The model under review builds one solid part; all positions refer to its coordinate system, in mm. A direction names the side the tool comes from. Round coordinates to 2 decimals unless told otherwise and drop trailing zeros. Write each loop counter-clockwise with the first axis right and the second up, starting at its lowest first coordinate (ties: lowest second). Pieces come first, ordered by that corner, then holes. Notation, with made-up numbers: (-6, 63.25) -> (6, 63.25) arc R28 cw to (6, 99.25) -> close; hole circle Ø7 at (80.25, 84). An arc over 180 degrees is marked (long way). Answer as a JSON object with one key per item and string values. Group by question number.
1) Machinability: for faces 5 (the cylindrical face through (68.476, -39.816, 4.336)), 6 (the cylindrical face through (55.99, -52.58, 16.85)), 7 (the cylindrical face through (4.056, 38.668, 5.077)), which of the approach directions +Z, -Z, +X, -X, +Y, -Y give a long, thin tool a straight path to every point of the face, cutting with its end or side? Answer none if there is none.
2) We need section C-C, the plane z = -29.5. Write out the cut boundary in (x, y).
3) Mouldability with a two-part tool opening along X and no side actions: class faces 1 (the cylindrical face through (55.844, -52.577, -16.716)), 2 (the cylindrical face through (75.31, -46.66, 2.82)), 3 (the cylindrical face through (132, -53, 0)), 4 (the flat face through (87, -47, 24)) as pulls with the +X half, pulls with the -X half, needs draft (parallel to the pull), parting line crosses it, or undercut.
4) We need section B-B, the plane x = 117. Write out the cut boundary in (y, z).
5) Insertion check: pin 1 Ø6 at (y, z) = (-30, 0) entering from -X; pin 2 Ø2 at (y, z) = (-43, -15) entering from +X; pin 3 Ø1.5 at (x, y) = (31, 12) entering from -Z. Each pin has a flat end and moves straight along its axis. Give the tip position at first contact, or say it passes through.
6) We need section D-D, the plane z = 0. Count the separate pieces of the cut face and the enclosed holes in it, then the cut area to 3 significant figures.
7) We need section A-A, the plane y = 30. Write out the cut boundary in (x, z).
8) To check wall thickness, follow probe 1 along Z at (x, y) = (88, -42.5); probe 2 along Y at (x, z) = (102, -19); probe 3 along Z at (x, y) = (94.5, -13). State the ranges of each line that lie inside material, in increasing order. Write a range as [from, to].
from build123d import *

# Parameters (mm, degrees)
PIPE_SECTION_SKETCH_40X_26_R        = 20
PIPE_SECTION_SKETCH_40X_26_R_2      = 13
ROUND_START                         = 8
ROUND_FLANGE_SKETCH_78_R            = 39
ROUND_FLANGE_SKETCH_78_R_2          = 13
ROUND_FLANGE_78_DEPTH               = 8
ROUND_FLANGE_BOLT_HOLES_4X_10_REACH = 130.643
ROUND_FLANGE_BOLT_HOLES_SKETCH_R    = 5
OVAL_FLANGE_SKETCH_R                = 6
OVAL_FLANGE_SKETCH_R_2              = 13
OVAL_FLANGE_DEPTH                   = 11
FLANGE_ROOT_FILLETS_R2_5_R          = 2.5


with BuildPart() as part:
    # Elbow Pipe Body: sweep along a path in Elbow Path Sketch
    with BuildLine(Plane.XY) as elbow_pipe_body_path:
        Line((0, 0), (53, 0))
        ThreePointArc((53, 0), (77.748737342, -10.251262658), (88, -35))
        Line((88, -35), (88, -58))
    # Pipe Section Sketch Ø40xØ26 → Elbow Pipe Body (sweep)
    with BuildSketch(Plane(origin=(0, 0, 0), x_dir=(0, 0, -1), z_dir=(1, 0, 0))):
        Circle(PIPE_SECTION_SKETCH_40X_26_R)
        Circle(PIPE_SECTION_SKETCH_40X_26_R_2, mode=Mode.SUBTRACT)
    sweep(path=elbow_pipe_body_path.line)

    # Round Flange Sketch Ø78 → Round Flange Ø78 (add)
    with BuildSketch(Plane(origin=(0, 0, 0), x_dir=(0, 0, -1), z_dir=(1, 0, 0)).offset(ROUND_START)):
        Circle(ROUND_FLANGE_SKETCH_78_R)
        with Locations(Location((0, 0, 0), (0, 0, 90))):
            Circle(ROUND_FLANGE_SKETCH_78_R_2, mode=Mode.SUBTRACT)
    extrude(amount=-ROUND_FLANGE_78_DEPTH)

    # Round Flange Bolt Holes Sketch → Round Flange Bolt Holes 4xØ10 (cut, up to next)
    with BuildSketch(Plane.ZY, mode=Mode.PRIVATE) as round_flange_bolt_holes_4x_10_sk1:
        with Locations((0, 30)):
            Circle(ROUND_FLANGE_BOLT_HOLES_SKETCH_R)
    round_flange_bolt_holes_4x_10_tool1 = extrude(round_flange_bolt_holes_4x_10_sk1.sketch, amount=-ROUND_FLANGE_BOLT_HOLES_4X_10_REACH, mode=Mode.PRIVATE) & part.part
    # Round Flange Bolt Holes Sketch → Round Flange Bolt Holes 4xØ10 (cut, up to next)
    with BuildSketch(Plane.ZY, mode=Mode.PRIVATE) as round_flange_bolt_holes_4x_10_sk2:
        with Locations((30, 0)):
            Circle(ROUND_FLANGE_BOLT_HOLES_SKETCH_R)
    round_flange_bolt_holes_4x_10_tool2 = extrude(round_flange_bolt_holes_4x_10_sk2.sketch, amount=-ROUND_FLANGE_BOLT_HOLES_4X_10_REACH, mode=Mode.PRIVATE) & part.part
    # Round Flange Bolt Holes Sketch → Round Flange Bolt Holes 4xØ10 (cut, up to next)
    with BuildSketch(Plane.ZY, mode=Mode.PRIVATE) as round_flange_bolt_holes_4x_10_sk3:
        with Locations((0, -30)):
            Circle(ROUND_FLANGE_BOLT_HOLES_SKETCH_R)
    round_flange_bolt_holes_4x_10_tool3 = extrude(round_flange_bolt_holes_4x_10_sk3.sketch, amount=-ROUND_FLANGE_BOLT_HOLES_4X_10_REACH, mode=Mode.PRIVATE) & part.part
    # Round Flange Bolt Holes Sketch → Round Flange Bolt Holes 4xØ10 (cut, up to next)
    with BuildSketch(Plane.ZY, mode=Mode.PRIVATE) as round_flange_bolt_holes_4x_10_sk4:
        with Locations((-30, 0)):
            Circle(ROUND_FLANGE_BOLT_HOLES_SKETCH_R)
    round_flange_bolt_holes_4x_10_tool4 = extrude(round_flange_bolt_holes_4x_10_sk4.sketch, amount=-ROUND_FLANGE_BOLT_HOLES_4X_10_REACH, mode=Mode.PRIVATE) & part.part
    add(round_flange_bolt_holes_4x_10_tool1.solids().sort_by_distance((0, 30, 0))[0], mode=Mode.SUBTRACT)
    add(round_flange_bolt_holes_4x_10_tool2.solids().sort_by_distance((0, 0, 30))[0], mode=Mode.SUBTRACT)
    add(round_flange_bolt_holes_4x_10_tool3.solids().sort_by_distance((0, -30, 0))[0], mode=Mode.SUBTRACT)
    add(round_flange_bolt_holes_4x_10_tool4.solids().sort_by_distance((0, 0, -30))[0], mode=Mode.SUBTRACT)

    # Oval Flange Sketch → Oval Flange (add)
    with BuildSketch(Plane.XZ.offset(58)):
        with BuildLine():
            ThreePointArc((60.803210464, -22.030311821), (88, -35), (115.196789536, -22.030311821))
            ThreePointArc((115.196789536, -22.030311821), (120.082146816, -16.784263387), (125.642563047, -12.259938988))
            ThreePointArc((125.642563047, -12.259938988), (132, 0), (125.642563047, 12.259938988))
            ThreePointArc((125.642563047, 12.259938988), (120.082146816, 16.784263387), (115.196789536, 22.030311821))
            ThreePointArc((115.196789536, 22.030311821), (88, 35), (60.803210464, 22.030311821))
            ThreePointArc((60.803210464, 22.030311821), (55.917853184, 16.784263387), (50.357436953, 12.259938988))
            ThreePointArc((50.357436953, 12.259938988), (44, 0), (50.357436953, -12.259938988))
            ThreePointArc((50.357436953, -12.259938988), (55.917853184, -16.784263387), (60.803210464, -22.030311821))
        make_face()
        with Locations((117, 0)):
            Circle(OVAL_FLANGE_SKETCH_R, mode=Mode.SUBTRACT)
        with Locations((59, 0)):
            Circle(OVAL_FLANGE_SKETCH_R, mode=Mode.SUBTRACT)
        with Locations(Location((88, 0, 0), (0, 0, 270))):
            Circle(OVAL_FLANGE_SKETCH_R_2, mode=Mode.SUBTRACT)
    extrude(amount=-OVAL_FLANGE_DEPTH)

    # Flange Root Fillets R2.5
    flange_root_fillets_r2_5_edges = [part.edges().sort_by_distance(p)[0] for p in [
        (8, 0, 20),
        (88, -47, 20),
    ]]
    fillet(flange_root_fillets_r2_5_edges, radius=FLANGE_ROOT_FILLETS_R2_5_R)


solid = part.part
Here are the results:
{
 "1": {"face 5": "none", "face 6": "+Z, -X, -Y", "face 7": "-X"},
 "2": {"outline": "(0, -25.51) -> (8, -25.51) -> (8, -4.97) -> (0, -4.97) -> close; (0, 4.97) -> (8, 4.97) -> (8, 25.51) -> (0, 25.51) -> close; (69.17, -58) -> (106.83, -58) -> (106.83, -47) -> (69.17, -47) -> close"},
 "3": {"face 1": "pulls with the -X half", "face 2": "undercut", "face 3": "pulls with the +X half", "face 4": "needs draft"},
 "4": {"outline": "(-58, -19.92) -> (-47, -19.92) -> (-47, -6) -> (-58, -6) -> close; (-58, 6) -> (-47, 6) -> (-47, 19.92) -> (-58, 19.92) -> close"},
 "5": {"pin 1": "stops at x = 65.69", "pin 2": "stops at x = 102.28", "pin 3": "stops at z = -16.54"},
 "6": {"separate pieces": "6", "enclosed holes": "0", "area": "2,250 mm^2"},
 "7": {"outline": "(0, -24.92) -> (8, -24.92) -> (8, -5) -> (0, -5) -> close; (0, 5) -> (8, 5) -> (8, 24.92) -> (0, 24.92) -> close"},
 "8": {"probe 1": "z = [-20, -13], [13, 20]", "probe 2": "y = [-58, -47]", "probe 3": "z = [-16.02, -5.07], [5.07, 16.02]"}
}
